Geometry check sheet. Reference: the model listing, model coordinates, mm. A direction names the side the tool comes from. Round coordinates to 2 decimals unless told otherwise and drop trailing zeros. Order: outer loops, then holes, each group sorted by start corner. A loop starts at its lowest first (then second) coordinate and runs counter-clockwise, first axis right, second up. Notation, with made-up numbers: (9, 26.5) - (17, 26.5) arc R19 ccw to (17, 40.5) - close; hole circle Ø11 at (37, -21.5). An arc over 180 degrees is marked (long way). Answer as CSV lines item,"result". Start each with the question number.
```python
from build123d import *

# Parameters (mm, degrees)
SKETCH1_W                                           = 36
SKETCH1_H                                           = 36
BOSS_EXTRUDE1_DEPTH                                 = 2.5
CBORE_FOR_M3_HEX_SOCKET_HEAD_CAP_SCREW1_D           = 3.4
CBORE_FOR_M3_HEX_SOCKET_HEAD_CAP_SCREW1_CBORE_D     = 6.5
CBORE_FOR_M3_HEX_SOCKET_HEAD_CAP_SCREW1_CBORE_DEPTH = 3.4
SKETCH5_R                                           = 11.5
CUT_EXTRUDE2_DEPTH                                  = 26.942243542


with BuildPart() as part:
    # Sketch1 → Boss-Extrude1 (new, symmetric)
    with BuildSketch(Plane(origin=(0, 0, 0), x_dir=(0, 0, -1), z_dir=(1, 0, 0))):
        Rectangle(SKETCH1_W, SKETCH1_H)
    extrude(amount=BOSS_EXTRUDE1_DEPTH, both=True)

    # CBORE for M3 Hex Socket Head Cap Screw1 (through all)
    with Locations(Plane(origin=(2.5, 0, 0), x_dir=(0, 0, -1), z_dir=(1, 0, 0))):
        with Locations((-14, 14), (14, 14), (-14, -14), (14, -14)):
            CounterBoreHole(CBORE_FOR_M3_HEX_SOCKET_HEAD_CAP_SCREW1_D / 2, CBORE_FOR_M3_HEX_SOCKET_HEAD_CAP_SCREW1_CBORE_D / 2, CBORE_FOR_M3_HEX_SOCKET_HEAD_CAP_SCREW1_CBORE_DEPTH)

    # Sketch5 → Cut-Extrude2 (cut, through all)
    with BuildSketch(Plane(origin=(2.5, 0, 0), x_dir=(0, 0, -1), z_dir=(1, 0, 0))):
        Circle(SKETCH5_R)
    extrude(amount=-CUT_EXTRUDE2_DEPTH, mode=Mode.SUBTRACT)


solid = part.part
```
1. Go/stop test with a flat-tipped pin: pin 1 Ø2 at (y, z) = (14.5, 15.5) entering from +X. Record where the tip stops, or that it passes through.
2. Section check C-C on x = -1.8. Record the boundary of the cut face in (y, z), plus the area to 3 significant figures.
3. Access from +Z, -Z, +X, -X, +Y, -Y to the whole of each face (thin tool, end or side, straight path). Record for faces 1 (the face through (0.824, -13.857, 17.247)), 2 (the face through (-1.71, 14.51, -12.38)).
4. Thickness scan on probe 1 along Y at (x, z) = (1.65, 14); probe 2 along Y at (x, z) = (-1.4, 14); probe 3 along Z at (x, y) = (-2.2, 15.5). Record the ranges inside material, lowest first.
5. Section check A-A on y = 0. Record the boundary of the cut face in (x, z).
6. Draft check along Z on faces 3 (the face through (0, 0, -18)), 4 (the face through (0.824, 14.143, 17.247)), 5 (the face through (0, 18, 0)). Enter one of: released by +Z, released by -Z, zero draft, split by the parting line, or undercut.
7. Section check D-D on y = -14. Record the boundary of the cut face in (x, z).
Numbers:
1,pin 1,"stops at x = -0.9"
2,outline,"(-18, -18) - (18, -18) - (18, 18) - (-18, 18) - close; hole circle Ø3.4 at (-14, -14); hole circle Ø3.4 at (-14, 14); hole circle Ø23 at (0, 0); hole circle Ø3.4 at (14, -14); hole circle Ø3.4 at (14, 14)"
2,area,"844 mm2"
3,face 1,"+X"
3,face 2,"+X, -X"
4,probe 1,"y = -18 to -17.25, -10.75 to 10.75, 17.25 to 18"
4,probe 2,"y = -18 to -15.7, -12.3 to 12.3, 15.7 to 18"
4,probe 3,"z = -18 to -14.8, -13.2 to 13.2, 14.8 to 18"
5,outline,"(-2.5, -18) - (2.5, -18) - (2.5, -11.5) - (-2.5, -11.5) - close; (-2.5, 11.5) - (2.5, 11.5) - (2.5, 18) - (-2.5, 18) - close"
6,face 3,"released by -Z"
6,face 4,"undercut"
6,face 5,"zero draft"
7,outline,"(-2.5, -18) - (2.5, -18) - (2.5, -17.25) - (-0.9, -17.25) - (-0.9, -15.7) - (-2.5, -15.7) - close; (-2.5, -12.3) - (-0.9, -12.3) - (-0.9, -10.75) - (2.5, -10.75) - (2.5, 10.75) - (-0.9, 10.75) - (-0.9, 12.3) - (-2.5, 12.3) - close; (-2.5, 15.7) - (-0.9, 15.7) - (-0.9, 17.25) - (2.5, 17.25) - (2.5, 18) - (-2.5, 18) - close"
